Input: part model. Units: mm. Frame: model coordinates. A direction names the side the tool comes from. Coordinates: 2 decimals unless noted, no trailing zeros. Order: outer loops, then holes, each group sorted by start corner. A loop starts at its lowest first (then second) coordinate and runs counter-clockwise, first axis right, second up. Notation, with made-up numbers: (6, 5) - (59, 5) arc R19 ccw to (59, 20) - close; hole circle Ø6 at (-26, 51.5). An arc over 180 degrees is marked (long way). One line per question, with ' | ' between items.
from build123d import *

# Parameters (mm, degrees)
BASE_BLOCK_DEPTH              = 60
TOP_SLOT_WITH_BORE_SEAT_DEPTH = 21
END_CHANNEL_PROFILE_W         = 30
END_CHANNEL_PROFILE_H         = 47.374117648
END_CHANNEL_CUT_DEPTH         = 180.69878471
TRIANGULAR_POCKET_CUT_DEPTH   = 40


with BuildPart() as part:
    # Base Block Profile → Base Block (new body)
    with BuildSketch(Plane.XY):
        Polygon((40, 28.687058824), (75, 28.687058824), (75, -28.687058824), (-75, -28.687058824), (-75, 28.687058824), (-40, 28.687058824), (-40, 78.687058824), (40, 78.687058824), align=None)
    extrude(amount=-BASE_BLOCK_DEPTH)

    # Top Slot Profile → Top Slot With Bore Seat (cut)
    with BuildSketch(Plane(origin=(0, 78.687058824, 0), x_dir=(1, 0, 0), z_dir=(0, 1, 0))):
        with BuildLine():
            Line((-40, 37.5), (-16.363068172, 37.5))
            ThreePointArc((-16.363068172, 37.5), (0, 48), (16.363068172, 37.5))
            Line((16.363068172, 37.5), (40, 37.5))
            Line((40, 37.5), (40, 22.5))
            Line((40, 22.5), (16.363068172, 22.5))
            ThreePointArc((16.363068172, 22.5), (0, 12), (-16.363068172, 22.5))
            Line((-16.363068172, 22.5), (-40, 22.5))
            Line((-40, 22.5), (-40, 37.5))
        make_face()
    extrude(amount=-TOP_SLOT_WITH_BORE_SEAT_DEPTH, mode=Mode.SUBTRACT)

    # End Channel Profile → End Channel Cut (cut, through all)
    with BuildSketch(Plane.ZY.offset(75)):
        with Locations((-29.740602956, 0)):
            Rectangle(END_CHANNEL_PROFILE_W, END_CHANNEL_PROFILE_H)
    extrude(amount=-END_CHANNEL_CUT_DEPTH, mode=Mode.SUBTRACT)

    # Triangular Pocket Profile → Triangular Pocket Cut (cut)
    with BuildSketch(Plane.XY.offset(-10)):
        Polygon((-48, 28.687058824), (-75, -28.687058824), (-75, 28.687058824), align=None)
        Polygon((48, 28.687058824), (75, -28.687058824), (75, 28.687058824), align=None)
    extrude(amount=-TRIANGULAR_POCKET_CUT_DEPTH, mode=Mode.SUBTRACT)


solid = part.part
Item 1: Ray query, line 1 (Y direction, x = 13, z = -34); line 2 (Z direction, x = -58, y = 9); line 3 (Z direction, x = -12, y = -22.5). Return the intervals inside material, ascending.
Data:
line 1: -28.69 to -23.69, 23.69 to 57.69 | line 2: -60 to -50, -10 to 0 | line 3: -60 to -44.74, -14.74 to 0
Item 2: Section D-D on z = -4.5. Return the cut outline in (x, y).
Data:
outline: (-75, -28.69) - (75, -28.69) - (75, 28.69) - (40, 28.69) - (40, 78.69) - (-40, 78.69) - (-40, 28.69) - (-75, 28.69) - close
Item 3: Contact query for flat-ended pins moving along their axis: P1, Ø1, axis at y = 41, z = -50, coming from the +X side; P2, Ø10.5, axis at x = -50, z = -27.5, coming from the +Y side; P3, Ø8, axis at y = 68, z = -52, coming from the -X side. Output: stop coordinate, or through.
Data:
P1: x = 40 | P2: y = 28.69 | P3: x = -40
Item 4: Draft query along Y for faces 1 (the face through (-67, 13, -50)), 2 (the face through (-1, 78.687, -49)), 3 (the face through (-1, -23.687, -30)). Return one class per face: released by +Y, released by -Y, zero draft, split by the parting line, or undercut.
Data:
face 1: zero draft | face 2: released by +Y | face 3: undercut
Item 5: Access query for faces 4 (the face through (1, 57.687, -30)), 5 (the face through (61.31, 0.4, -11.94)), 6 (the face through (-28, 68, -37.5)). Directions: +Z, -Z, +X, -X, +Y, -Y. A direction counts if a zero-diameter tool reaches every point of the face in a straight line with its end or side. Return the directions, or none.
Data:
face 4: +Y | face 5: +X, +Y | face 6: +X, -X, +Y
Item 6: Section C-C on y = 5.5. Return the cut outline in (x, z), and give its area (3 significant figures).
Data:
outline: (-75, -60) - (75, -60) - (75, -50) - (58.91, -50) - (58.91, -44.74) - (-58.91, -44.74) - (-58.91, -50) - (-75, -50) - close; (-75, -10) - (-58.91, -10) - (-58.91, -14.74) - (58.91, -14.74) - (58.91, -10) - (75, -10) - (75, 0) - (-75, 0) - close | area: 4,180 mm^2
Item 7: Section B-B on x = 28.5. Return the cut outline in (y, z).
Data:
outline: (-28.69, -60) - (78.69, -60) - (78.69, -37.5) - (57.69, -37.5) - (57.69, -22.5) - (78.69, -22.5) - (78.69, 0) - (-28.69, 0) - close; hole (-23.69, -44.74) - (23.69, -44.74) - (23.69, -14.74) - (-23.69, -14.74) - close
Item 8: Section A-A on z = -25.5. Return the cut outline in (x, y).
Data:
outline: (-75, -28.69) - (75, -28.69) - (72.65, -23.69) - (-72.65, -23.69) - close; (-50.35, 23.69) - (50.35, 23.69) - (48, 28.69) - (40, 28.69) - (40, 57.69) - (-40, 57.69) - (-40, 28.69) - (-48, 28.69) - close
